```python
from build123d import *

# Parameters (mm, degrees)
SKETCH1_W             = 100
SKETCH1_H             = 100
BOSS_EXTRUDE1_DEPTH   = 2000
FILLET1_R             = 8.4
SHELL1_T              = -4
M8_TAPPED_HOLE1_D     = 6.8
M8_TAPPED_HOLE1_DEPTH = 19.75
M8_TAPPED_HOLE1_TIP   = 2.042926105
SKETCH2_R             = 7.5
SKETCH2_R_2           = 3
CUT_EXTRUDE1_DEPTH    = 10


with BuildPart() as part:
    # Sketch1 → Boss-Extrude1 (new body)
    with BuildSketch(Plane.XY):
        Rectangle(SKETCH1_W, SKETCH1_H)
    extrude(amount=BOSS_EXTRUDE1_DEPTH)

    # Fillet1
    fillet1_edges = [part.edges().sort_by_distance(p)[0] for p in [
        (-50, 50, 1000),
        (50, 50, 1000),
        (50, -50, 1000),
        (-50, -50, 1000),
    ]]
    fillet(fillet1_edges, radius=FILLET1_R)

    # Shell1
    shell1_openings = [part.faces().sort_by_distance(p)[0] for p in [
        (0, 0, 2000),
        (0, 0, 0),
    ]]
    offset(amount=SHELL1_T, openings=shell1_openings, kind=Kind.INTERSECTION)

    # M8 Tapped Hole1
    with Locations(Plane(origin=(0, 50, 0), x_dir=(1, 0, 0), z_dir=(0, 1, 0))):
        with Locations((-35, -390), (35, -390), (35, -480), (-35, -480)):
            Hole(M8_TAPPED_HOLE1_D / 2, depth=M8_TAPPED_HOLE1_DEPTH)
            with Locations((0, 0, -(M8_TAPPED_HOLE1_DEPTH + M8_TAPPED_HOLE1_TIP / 2))):  # 118° drill point
                Cone(0, M8_TAPPED_HOLE1_D / 2, M8_TAPPED_HOLE1_TIP, mode=Mode.SUBTRACT)

    # Sketch2 → Cut-Extrude1 (cut)
    with BuildSketch(Plane(origin=(0, 50, 0), x_dir=(1, 0, 0), z_dir=(0, 1, 0))):
        with Locations(Location((35, -618, 0), (0, 0, 331.642363424))):
            Circle(SKETCH2_R)
        with Locations(Location((-35, -618, 0), (0, 0, 208.357636576))):
            Circle(SKETCH2_R)
        with Locations(Location((35, -1382, 0), (0, 0, 331.642363424))):
            Circle(SKETCH2_R)
        with Locations(Location((-35, -1382, 0), (0, 0, 208.357636576))):
            Circle(SKETCH2_R)
        with Locations((-35, -390)):
            Circle(SKETCH2_R_2)
        with Locations((35, -390)):
            Circle(SKETCH2_R_2)
        with Locations((35, -480)):
            Circle(SKETCH2_R_2)
        with Locations((-35, -480)):
            Circle(SKETCH2_R_2)
    extrude(amount=-CUT_EXTRUDE1_DEPTH, mode=Mode.SUBTRACT)


solid = part.part
```
For this review, take the finished solid that the model builds, in its own axes (mm). A direction names the side the tool comes from. Round coordinates to 2 decimals unless told otherwise and drop trailing zeros. Write each loop counter-clockwise with the first axis right and the second up, starting at its lowest first coordinate (ties: lowest second). Pieces come first, ordered by that corner, then holes. Notation, with made-up numbers: (-11, -13.75) -> (35, -13.75) arc R22 ccw to (35, 19.25) -> close; hole circle Ø7 at (-12.75, 78). An arc over 180 degrees is marked (long way). Use one line per item in the form item = value.
Q1. Clearance check with a flat-ended pin moving along its axis: pin 1 Ø9 at (x, z) = (-35, 618) entering from +Y. State where the tip first meets the part, or that it passes through.
Resolved:
pin_1 = -46
Q2. Machinability: for faces 1 (the flat face through (0, 48, 0)), 2 (the flat face through (-46, -1, 986)), which of the approach directions +Z, -Z, +X, -X, +Y, -Y give a long, thin tool a straight path to every point of the face, cutting with its end or side? Answer none if there is none.
Resolved:
face_1 = -Z, +X, -X, +Y, -Y
face_2 = +Z, -Z
Q3. The part is to be moulded in two halves that separate along X. For faces 3 (the flat face through (-1, -50, 986)), 4 (the flat face through (-1, 46, 986)), 5 (the flat face through (50, -1, 986)), 6 (the flat face through (-50, -1, 986)), say which applies: released by +X, released by -X, zero draft, split by the parting line, or undercut.
Resolved:
face_3 = zero draft
face_4 = undercut
face_5 = released by +X
face_6 = released by -X
Q4. Consider section A-A (z = 1838). State the section outline as (x, y) points.
Resolved:
outline = (-50, -41.6) arc R8.4 ccw to (-41.6, -50) -> (41.6, -50) arc R8.4 ccw to (50, -41.6) -> (50, 41.6) arc R8.4 ccw to (41.6, 50) -> (-41.6, 50) arc R8.4 ccw to (-50, 41.6) -> close; hole (-46, -41.6) arc R4.4 ccw to (-41.6, -46) -> (41.6, -46) arc R4.4 ccw to (46, -41.6) -> (46, 41.6) arc R4.4 ccw to (41.6, 46) -> (-41.6, 46) arc R4.4 ccw to (-46, 41.6) -> close
Q5. To check wall thickness, follow probe 1 along Z at (x, y) = (-35, 47.5); probe 2 along Y at (x, z) = (19, 100). State the ranges of each line that lie inside material, in increasing order. Write a range as from..to.
Resolved:
probe_1 = 0..386.6, 393.4..476.6, 483.4..610.5, 625.5..1374.5, 1389.5..2000
probe_2 = -50..-46, 46..50
